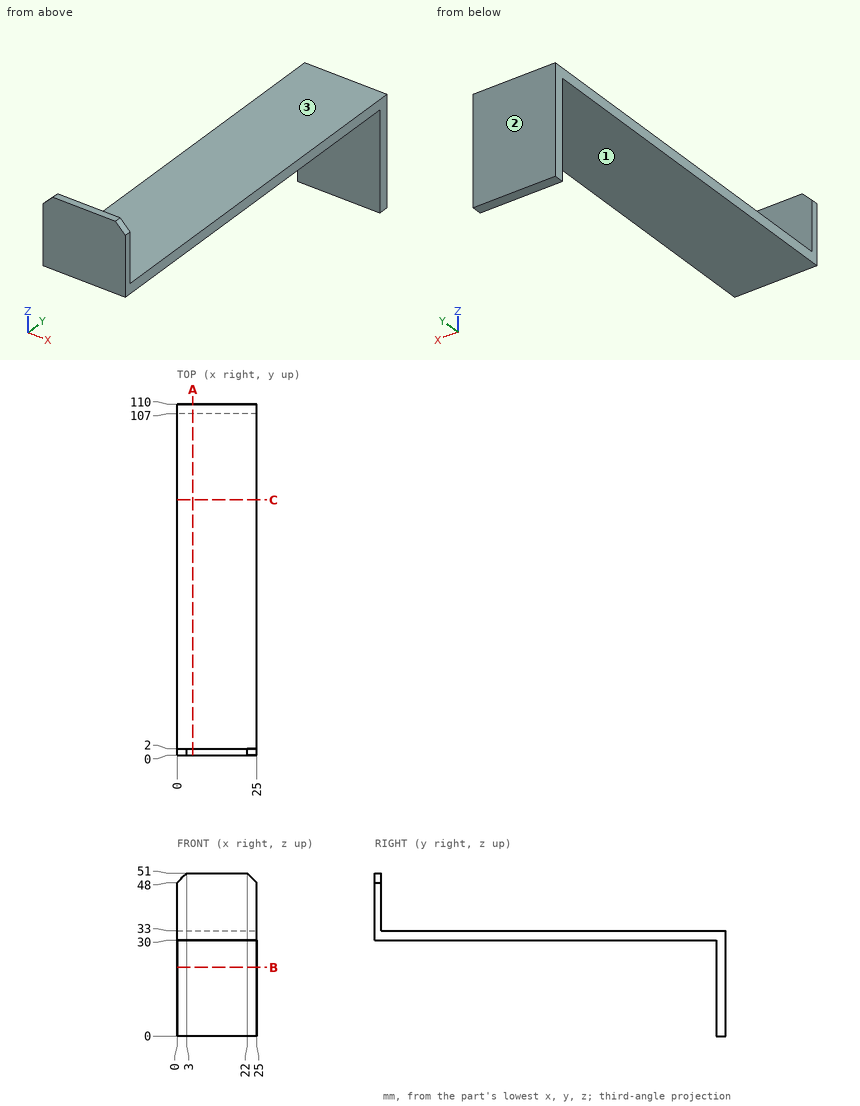
Answer from the drawing. Dimensions are ordinates in mm from the lowest x, y and z of the part. A direction names the side the tool comes from. Coordinates: 2 decimals unless noted, no trailing zeros. Order: outer loops, then holes, each group sorted by start corner. A loop starts at its lowest first (then second) coordinate and runs counter-clockwise, first axis right, second up. Notation, with made-up numbers: M -24.5,-37 L 30.5,-37 A17 cw 30.5,-21 Z; hole C 55,-31.5 d4. An arc over 180 degrees is marked long. Put each result on its own line as item: value. Start each with the question number.
Item 1: Section A-A, the plane x = 5 is taken. Determine the outline of the cut face in (y, z), plus the area to 3 significant figures.
Item 2: For the marked faces 1, 2 and 3, determine the directions among +Z, -Z, +X, -X, +Y, -Y from which every point of the face is accessible in a straight line to the end or side of a thin tool.
Item 3: Section C-C, the plane y = 80 is taken. Determine the outline of the cut face in (x, z).
Item 4: Given pin 1 Ø2 at (x, z) = (19.5, 21) entering from -Y; pin 2 Ø12.5 at (x, y) = (10, 50) entering from -Z; pin 3 Ø9 at (x, z) = (11, 45) entering from +Y, each flat-ended and moving along its own axis, determine where each tip first touches the part or whether it passes through.
Item 5: Consider probe 1 along Y at (x, z) = (8, 45); probe 2 along Y at (x, z) = (4, 6.5); probe 3 along Z at (x, y) = (19.25, 33.5). Determine where each line is inside the solid, lowest interval first. Write a range as [from, to].
Item 6: Section B-B, the plane z = 21.5 is taken. Determine the outline of the cut face in (x, y).
Computed:
1. outline: M 0,30 L 107,30 L 107,0 L 110,0 L 110,33 L 2,33 L 2,51 L 0,51 Z
1. area: 456 mm2
2. face 1: -Z, +X, -X, -Y
2. face 2: +Z, -Z, +X, -X, +Y
2. face 3: +Z, +X, -X, +Y
3. outline: M 0,30 L 25,30 L 25,33 L 0,33 Z
4. pin 1: stops at y = 107
4. pin 2: stops at z = 30
4. pin 3: stops at y = 2
5. probe 1: y = [0, 2]
5. probe 2: y = [107, 110]
5. probe 3: z = [30, 33]
6. outline: M 0,107 L 25,107 L 25,110 L 0,110 Z
